```python
from build123d import *

# Parameters (mm, degrees)
PATTERN_LINEAR_1_COUNT      = 2
PATTERN_LINEAR_1_PITCH      = 20.506096654
PATTERN_LINEAR_1_COUNT_DIR2 = 2
PATTERN_LINEAR_1_PITCH_DIR2 = 20.506096654


with BuildPart() as part:
    # 草图1 → 旋转1 (revolve)
    with BuildSketch(Plane.XY, mode=Mode.PRIVATE) as revolve_1_sk:
        with BuildLine():
            Line((0, 20), (0, 5))
            Line((0, 5), (29, 5))
            Line((29, 5), (29, 8.55))
            ThreePointArc((29, 8.55), (28.721751442, 9.221751442), (28.05, 9.5))
            Line((28.05, 9.5), (7, 9.5))
            Line((7, 9.5), (7, 9.2))
            Line((7, 9.2), (6, 9.2))
            Line((6, 9.2), (6, 20))
            Line((6, 20), (0, 20))
        make_face()
    revolve(revolve_1_sk.sketch.rotate(Axis((29, 0, 0), (-1, 0, 0)), 270), axis=Axis((29, 0, 0), (-1, 0, 0)))

    # 草图2 → 切除-旋转1 (revolve, cut)
    with BuildSketch(Plane.XY, mode=Mode.PRIVATE) as cut_revolve_1_sk:
        Polygon((0, 14.5), (0, 18.25), (4.1, 18.25), (4.1, 16.75), (6, 16.75), (6, 14.5), align=None)
    cut_revolve_1 = revolve(cut_revolve_1_sk.sketch.rotate(Axis((6, 14.5, 0), (-1, 0, 0)), 270), axis=Axis((6, 14.5, 0), (-1, 0, 0)), mode=Mode.SUBTRACT)

    # 阵列(线性)1: Cut-Revolve 1 2 × 2
    with Locations(*[Vector(0, -0.7071067811865475, 0.7071067811865477) * (i * PATTERN_LINEAR_1_PITCH) + Vector(0, -0.7071067811865477, -0.7071067811865474) * (j * PATTERN_LINEAR_1_PITCH_DIR2) for i in range(PATTERN_LINEAR_1_COUNT) for j in range(PATTERN_LINEAR_1_COUNT_DIR2) if (i, j) != (0, 0)]):
        add(cut_revolve_1, mode=Mode.SUBTRACT)


solid = part.part
```
Input: part model. Units: mm. Frame: model coordinates. A direction names the side the tool comes from. Give positions to 0.01 mm unless a question says otherwise; leave off trailing zeros. Order: outer loops, then holes, each group sorted by start corner. A loop starts at its lowest first (then second) coordinate and runs counter-clockwise, first axis right, second up.
1. Line query: probe 1 along Y at (x, z) = (0.9, 0); probe 2 along Y at (x, z) = (5.3, 0); probe 3 along X at (y, z) = (-13, -2.5). Output: solid intervals per line, ascending.
Computed:
probe 1: y = -20 to -18.25, -10.75 to -5, 5 to 10.75, 18.25 to 20
probe 2: y = -20 to -16.75, -12.25 to -5, 5 to 12.25, 16.75 to 20
probe 3: x = 4.1 to 6
2. Cut plane A-A (y = 0). State how many separate pieces and enclosed holes the cut face has, and give its area (3 significant figures).
Computed:
separate pieces: 4
enclosed holes: 0
area: 307 mm2
3. Pin query (flat end, axial travel): pin 1 Ø6 at (y, z) = (0, 14.5) entering from -X; pin 2 Ø3 at (x, y) = (21.5, 7) entering from -Z; pin 3 Ø6 at (y, z) = (0, -14.5) entering from +X. Return the tip coordinate at first contact, or that it passes through.
Computed:
pin 1: stops at x = 4.1
pin 2: stops at z = -7.75
pin 3: stops at x = 6
4. Set-up query: faces 1 (the face through (4.1, -2, -13)), 2 (the face through (17.38, -5.78, -7.54)), 3 (the face through (0, -4, 4)). Return all of +Z, -Z, +X, -X, +Y, -Y with unobstructed straight access to the full face (end or side cutting, diameter ignored); none if empty.
Computed:
face 1: -X
face 2: +X
face 3: +Z, -Z, -X, +Y, -Y
5. Cut plane D-D (y = -13). Return loops of the section in (x, z), and give its area (3 significant figures).
Computed:
outline: (0, -15.2) - (6, -15.2) - (6, -1.68) - (4.1, -1.68) - (4.1, -3.44) - (0, -3.44) - close; (0, 3.44) - (4.1, 3.44) - (4.1, 1.68) - (6, 1.68) - (6, 15.2) - (0, 15.2) - close
area: 148 mm2
6. Draft query along X for faces 4 (the face through (4.1, -2, 16)), 5 (the face through (2.08, -18.16, -0.81)), 6 (the face through (6.493, 2.763, 8.775)). Return one class per face: released by +X, released by -X, zero draft, split by the parting line, or undercut.
Computed:
face 4: released by -X
face 5: zero draft
face 6: undercut
7. Cut plane C-C (z = 14.5). Return loops of the section in (x, y).
Computed:
outline: (0, -13.77) - (6, -13.77) - (6, -2.25) - (4.1, -2.25) - (4.1, -3.75) - (0, -3.75) - close; (0, 3.75) - (4.1, 3.75) - (4.1, 2.25) - (6, 2.25) - (6, 13.77) - (0, 13.77) - close
